```python
from build123d import *

# Parameters (mm, degrees)
BASE_PLATE_DEPTH        = 10
MOUNTING_HOLES_SKETCH_R = 6
MOUNTING_HOLES_4X_DEPTH = 10
SLOT_BOSS_DEPTH         = 20
SLOT_THROUGH_CUT_DEPTH  = 20
BACK_CHANNEL_CUT_DEPTH  = 60


with BuildPart() as part:
    # Base Plate Sketch → Base Plate (new body)
    with BuildSketch(Plane.XY):
        with BuildLine():
            Line((15, 0), (85, 0))
            ThreePointArc((85, 0), (95.606601718, -4.393398282), (100, -15))
            Line((100, -15), (100, -45))
            ThreePointArc((100, -45), (95.606601718, -55.606601718), (85, -60))
            Line((85, -60), (15, -60))
            ThreePointArc((15, -60), (4.393398282, -55.606601718), (0, -45))
            Line((0, -45), (0, -15))
            ThreePointArc((0, -15), (4.393398282, -4.393398282), (15, 0))
        make_face()
    extrude(amount=BASE_PLATE_DEPTH)

    # Mounting Holes Sketch → Mounting Holes 4x (cut)
    with BuildSketch(Plane.XY.offset(10)):
        with Locations((15, -15)):
            Circle(MOUNTING_HOLES_SKETCH_R)
        with Locations((85, -15)):
            Circle(MOUNTING_HOLES_SKETCH_R)
        with Locations((85, -45)):
            Circle(MOUNTING_HOLES_SKETCH_R)
        with Locations((15, -45)):
            Circle(MOUNTING_HOLES_SKETCH_R)
    extrude(amount=-MOUNTING_HOLES_4X_DEPTH, mode=Mode.SUBTRACT)

    # Slot Boss Sketch → Slot Boss (add)
    with BuildSketch(Plane.XY.offset(10)):
        with BuildLine():
            Line((37.5, -16), (62.5, -16))
            ThreePointArc((62.5, -16), (76.5, -30), (62.5, -44))
            Line((62.5, -44), (37.5, -44))
            ThreePointArc((37.5, -44), (23.5, -30), (37.5, -16))
        make_face()
    extrude(amount=SLOT_BOSS_DEPTH)

    # Slot Cut Sketch → Slot Through Cut (cut)
    with BuildSketch(Plane.XY.offset(30)):
        with BuildLine():
            Line((37.5, -23), (62.5, -23))
            ThreePointArc((62.5, -23), (69.5, -30), (62.5, -37))
            Line((62.5, -37), (37.5, -37))
            ThreePointArc((37.5, -37), (30.5, -30), (37.5, -23))
        make_face()
    extrude(amount=-SLOT_THROUGH_CUT_DEPTH, mode=Mode.SUBTRACT)

    # Back Channel Sketch → Back Channel Cut (cut)
    with BuildSketch(Plane.XZ.offset(60)):
        Polygon((50, 0), (67.5, 0), (67.5, 5), (32.5, 5), (32.5, 0), align=None)
    extrude(amount=-BACK_CHANNEL_CUT_DEPTH, mode=Mode.SUBTRACT)


solid = part.part
```
For this review, take the finished solid that the model builds, in its own axes (mm). A direction names the side the tool comes from. Round coordinates to 2 decimals unless told otherwise and drop trailing zeros. Loops run counter-clockwise (first coordinate to the right, second up) from the corner with the lowest first, then second, coordinate; pieces in that order, holes last.
(1) Mouldability with a two-part tool opening along Y and no side actions: class faces 1 (the cylindrical face through (30.5, -30.15, 20.14)), 2 (the flat face through (50, -30, 5)), 3 (the flat face through (50, 0, 6)), 4 (the cylindrical face through (95.72, -55.49, 4.93)) as released by +Y, released by -Y, zero draft, split by the parting line, or undercut.
Returned:
face 1: undercut
face 2: zero draft
face 3: released by +Y
face 4: released by -Y
(2) We need section D-D (y = -30). Give the boundary of the cut face in (x, z), plus the area to 4 significant figures.
Returned:
outline: (0, 0) - (32.5, 0) - (32.5, 5) - (67.5, 5) - (67.5, 0) - (100, 0) - (100, 10) - (76.5, 10) - (76.5, 30) - (69.5, 30) - (69.5, 10) - (30.5, 10) - (30.5, 30) - (23.5, 30) - (23.5, 10) - (0, 10) - close
area: 1,105 mm2
(3) Tool access review of faces 5 (the flat face through (50, -37, 20)), 6 (the flat face through (32.5, -30, 3)), 7 (the cylindrical face through (76.497, -29.692, 19.86)), 8 (the flat face through (50, -16, 20)): name each direction out of +Z, -Z, +X, -X, +Y, -Y from which nothing blocks a thin tool from reaching the whole face with its end or side.
Returned:
face 5: +Z
face 6: -Z, +Y, -Y
face 7: +Z, +X
face 8: +Z, +X, -X, +Y
(4) Wall thickness on line 1 along Y through (x, z) = (85, 7); line 2 along X through (y, z) = (-30.5, 26.5); line 3 along Y through (x, z) = (60, 17.75): over which ranges is each line inside the solid? List them lowest first.
Returned:
line 1: y = -60 to -51, -39 to -21, -9 to 0
line 2: x = 23.51 to 30.52, 69.48 to 76.49
line 3: y = -44 to -37, -23 to -16
(5) Clearance check with flat-ended pins moving along their axes: P1, Ø17.5, axis at x = 44, y = -32.5, coming from the -Z side; P2, Ø11, axis at x = 85, y = -45, coming from the -Z side; P3, Ø10, axis at x = 55, z = 16, coming from the -Y side; P4, Ø19, axis at x = 15, y = -15, coming from the +Z side. State where each tip first meets the part, or that it passes through.
Returned:
P1: stops at z = 5
P2: passes through
P3: stops at y = -44
P4: stops at z = 10
(6) We need section A-A (z = 8). Give the boundary of the cut face in (x, y).
Returned:
outline: (0, -45) arc R15 ccw to (15, -60) - (85, -60) arc R15 ccw to (100, -45) - (100, -15) arc R15 ccw to (85, 0) - (15, 0) arc R15 ccw to (0, -15) - close; hole circle Ø12 at (15, -45); hole circle Ø12 at (15, -15); hole circle Ø12 at (85, -45); hole circle Ø12 at (85, -15)
(7) We need section B-B (x = 45). Give the boundary of the cut face in (y, z), plus the area to 3 significant figures.
Returned:
outline: (-60, 5) - (0, 5) - (0, 10) - (-16, 10) - (-16, 30) - (-23, 30) - (-23, 10) - (-37, 10) - (-37, 30) - (-44, 30) - (-44, 10) - (-60, 10) - close
area: 580 mm2
(8) We need section C-C (z = 19). Give the boundary of the cut face in (x, y), plus the area to 3 significant figures.
Returned:
outline: (37.5, -44) - (62.5, -44) arc R14 ccw to (62.5, -16) - (37.5, -16) arc R14 ccw to start; hole (37.5, -37) - (62.5, -37) arc R7 ccw to (62.5, -23) - (37.5, -23) arc R7 ccw to start
area: 812 mm2
